Part model, mm, in its own coordinate system. A direction names the side the tool comes from. Round coordinates to 2 decimals unless told otherwise and drop trailing zeros. Order: outer loops, then holes, each group sorted by start corner. A loop starts at its lowest first (then second) coordinate and runs counter-clockwise, first axis right, second up. Notation, with made-up numbers: (46.25, 20.25) - (96.25, 20.25) arc R26 cw to (96.25, 36.25) - close; hole circle Ø11 at (-6, 23.5). An arc over 180 degrees is marked (long way). Return JSON: item names as keys, results as strings. Group by question number.
Item 1: Saw through at D-D on z = 3.5. List the corners of the cut face in (x, y).
Item 2: Saw through at A-A on x = 23. List the corners of the cut face in (y, z).
Item 3: Drop flat-ended pins along their axis: pin 1 (5.5 mm diameter, centred on x = 7.5, z = 4, fed in from +Y); pin 2 (1 mm diameter, centred on x = 26, z = 5, fed in from -Y). Give the stop position or say it passes through.
Item 4: Saw through at B-B on y = 22. List the corners of the cut face in (x, z).
Item 5: Probe probe 1 along Z at (x, y) = (8, 25.25); probe 2 along X at (y, z) = (20.5, 2); probe 3 along X at (y, z) = (4.5, 4). List the from-to ranges inside material, lowest first.
Item 6: Saw through at C-C on y = 15.5. List the corners of the cut face in (x, z), and give its area (3 significant figures).
Item 7: Two-plate mould, pull along Z, no slides. Class faces 3 (the face through (0, 15, 6)), 4 (the face through (1, 15, 1)), 5 (the face through (35.6, 13.6, 8.4)): released by +Z, released by -Z, zero draft, split by the parting line, or undercut.
Item 8: Tool access for faces 1 (the face through (23, 30, 6)), 2 (the face through (42.85, 21.91, 8.59)): list every direction of +Z, -Z, +X, -X, +Y, -Y with a clear straight run to the whole face (end or side of a thin tool).
```python
from build123d import *

# Parameters (mm, degrees)
SKETCH_1_W                   = 46
SKETCH_1_H                   = 30
EXTRUDE_1_DEPTH              = 12
HOLE_WIZARD_7_0_7_1_D        = 7
HOLE_WIZARD_M6_1_D           = 6.4
HOLE_WIZARD_M6_1_CBORE_D     = 11
HOLE_WIZARD_M6_1_CBORE_DEPTH = 6.4
SKETCH_7_R                   = 5.5
CUT_EXTRUDE_1_DEPTH          = 10
CHAMFER_1_SIZE               = 2


with BuildPart() as part:
    # 草图1 → 凸台-拉伸1 (new body)
    with BuildSketch(Plane.XY):
        with Locations((23, 15)):
            Rectangle(SKETCH_1_W, SKETCH_1_H)
    extrude(amount=EXTRUDE_1_DEPTH)

    # Ø7.0 (7) 直径孔1 (through all)
    with Locations(Plane.XY.offset(12)):
        with Locations((23, 22)):
            Hole(HOLE_WIZARD_7_0_7_1_D / 2)

    # M6 六角凹头螺钉的柱形沉头孔1 (through all)
    with Locations(Plane(origin=(0, 30, 0), x_dir=(1, 0, 0), z_dir=(0, 1, 0))):
        with Locations((8, -6), (38, -6)):
            CounterBoreHole(HOLE_WIZARD_M6_1_D / 2, HOLE_WIZARD_M6_1_CBORE_D / 2, HOLE_WIZARD_M6_1_CBORE_DEPTH)

    # 草图7 → 切除-拉伸1 (cut)
    with BuildSketch(Plane(origin=(0, 23.6, 0), x_dir=(1, 0, 0), z_dir=(0, 1, 0))):
        with Locations(Location((8, -6, 0), (0, 0, 270))):
            Circle(SKETCH_7_R)
        with Locations(Location((38, -6, 0), (0, 0, 270))):
            Circle(SKETCH_7_R)
    extrude(amount=-CUT_EXTRUDE_1_DEPTH, mode=Mode.SUBTRACT)

    # 倒角1
    chamfer_1_edges = [part.edges().sort_by_distance(p)[0] for p in [
        (46, 15, 12),
        (0, 15, 12),
        (46, 15, 0),
        (0, 15, 0),
    ]]
    chamfer(chamfer_1_edges, length=CHAMFER_1_SIZE)


solid = part.part
```
Filled in:
{
 "1": {"outline": "(0, 0) - (6, 0) - (6, 13.6) - (3.1, 13.6) - (3.1, 30) - (0, 30) - close; (10, 0) - (36, 0) - (36, 13.6) - (33.1, 13.6) - (33.1, 30) - (12.9, 30) - (12.9, 13.6) - (10, 13.6) - close; (40, 0) - (46, 0) - (46, 30) - (42.9, 30) - (42.9, 13.6) - (40, 13.6) - close; hole circle Ø7 at (23, 22)"},
 "2": {"outline": "(0, 0) - (18.5, 0) - (18.5, 12) - (0, 12) - close; (25.5, 0) - (30, 0) - (30, 12) - (25.5, 12) - close"},
 "3": {"pin 1": "stops at y = 13.6", "pin 2": "stops at y = 0"},
 "4": {"outline": "(0, 2) - (2, 0) - (19.5, 0) - (19.5, 12) - (2, 12) - (0, 10) - close; (26.5, 0) - (44, 0) - (46, 2) - (46, 10) - (44, 12) - (26.5, 12) - close; hole circle Ø11 at (8, 6); hole circle Ø11 at (38, 6)"},
 "5": {"probe 1": "z = 0 to 0.5, 11.5 to 12", "probe 2": "x = 0 to 4.23, 11.77 to 19.84, 26.16 to 34.23, 41.77 to 46", "probe 3": "x = 0 to 5.5, 10.5 to 35.5, 40.5 to 46"},
 "6": {"outline": "(0, 2) - (2, 0) - (44, 0) - (46, 2) - (46, 10) - (44, 12) - (2, 12) - (0, 10) - close; hole circle Ø11 at (8, 6); hole circle Ø11 at (38, 6)", "area": "354 mm^2"},
 "7": {"face 3": "zero draft", "face 4": "released by -Z", "face 5": "undercut"},
 "8": {"face 1": "+Z, -Z, +X, -X, +Y", "face 2": "+Y"}
}
